```python
from build123d import *

# Parameters (mm, degrees)
SKETCH1_R           = 3
BOSS_EXTRUDE1_DEPTH = 25
FILLET1_R           = 20


with BuildPart() as part:
    # Sketch1 → Boss-Extrude1 (new body)
    with BuildSketch(Plane(origin=(0, 0, 0), x_dir=(1, 0, 0), z_dir=(0, 1, 0))):
        Polygon((67.5, 0), (0, 0), (0, -394.016321232), (67.5, -314.016321232), align=None)
        with Locations(Location((33.75, -315.248874166, 0), (0, 0, 270))):
            Circle(SKETCH1_R, mode=Mode.SUBTRACT)
    extrude(amount=BOSS_EXTRUDE1_DEPTH)

    # Fillet1
    fillet1_edges = [part.edges().sort_by_distance(p)[0] for p in [
        (0, 12.5, 0),
    ]]
    fillet(fillet1_edges, radius=FILLET1_R)


solid = part.part
```
Work out the finished part from the listing and answer in its coordinate system (mm). Coordinates: 2 decimals unless noted, no trailing zeros. Write each loop counter-clockwise with the first axis right and the second up, starting at its lowest first coordinate (ties: lowest second). Pieces come first, ordered by that corner, then holes. Notation, with made-up numbers: (88.5, -4.5) - (98.5, -4.5) arc R6 cw to (98.5, 5.5) - close; hole circle Ø9 at (35.5, 4). An arc over 180 degrees is marked (long way). Answer as a JSON object with one key per item and string values.
Q1. Given pin 1 Ø12 at (x, y) = (13.5, 20.5) entering from -Z; pin 2 Ø8 at (x, y) = (12, 8) entering from +Z; pin 3 Ø1 at (x, y) = (38.5, 6) entering from +Z, each flat-ended and moving along its own axis, determine where each tip first touches the part or whether it passes through.
Results list:
{"pin 1": "stops at z = 0.01", "pin 2": "stops at z = 384.53", "pin 3": "stops at z = 348.98"}
Q2. Find section B-B (x = 12.5). Write down the section's boundary in (y, z), plus the area to 3 significant figures.
Results list:
{"outline": "(0, 1.46) - (25, 1.46) - (25, 379.2) - (0, 379.2) - close", "area": "9,440 mm^2"}
Q3. Find section A-A (y = 10.25). Write down the section's boundary in (x, z), plus the area to 3 significant figures.
Results list:
{"outline": "(0, 20) arc R20 ccw to (20, 0) - (67.5, 0) - (67.5, 314.02) - (0, 394.02) - close; hole circle Ø6 at (33.75, 315.25)", "area": "23,800 mm^2"}
Q4. Consider L1, parallel to Z at x = 33.5, y = 19.5; L2, parallel to Z at x = 13.5, y = 14; L3, parallel to Z at x = 6, y = 11. Determine where each line is inside the solid, lowest interval first. Write a range as from..to.
Results list:
{"L1": "z = 0..312.26, 318.24..354.31", "L2": "z = 1.09..378.02", "L3": "z = 5.72..386.91"}
Q5. Find section C-C (z = 336.5). Write down the section's boundary in (x, y), plus the area to 3 significant figures.
Results list:
{"outline": "(0, 0) - (48.53, 0) - (48.53, 25) - (0, 25) - close", "area": "1,210 mm^2"}
